from build123d import *

# Parameters (mm, degrees)
EXTRUDE1_DEPTH        = 78
M5_TAPPED_HOLE1_D     = 4.2
M5_TAPPED_HOLE1_DEPTH = 14.4
M5_TAPPED_HOLE1_TIP   = 1.2618073
SKETCH3_R             = 2.75
CUT_EXTRUDE1_DEPTH    = 93.649878575


with BuildPart() as part:
    # Sketch1 → Extrude1 (new, symmetric)
    with BuildSketch(Plane.XY):
        Polygon((0, 55), (0, 0), (30, 0), (30, 15), (15, 15), (15, 55), align=None)
    extrude(amount=EXTRUDE1_DEPTH, both=True)

    # M5 Tapped Hole1
    with Locations(Plane(origin=(7.5, 55, 0), x_dir=(0, 0, 1), z_dir=(0, 1, 0))):
        with Locations((0, 0), (-70, 0), (70, 0)):
            Hole(M5_TAPPED_HOLE1_D / 2, depth=M5_TAPPED_HOLE1_DEPTH)
            with Locations((0, 0, -(M5_TAPPED_HOLE1_DEPTH + M5_TAPPED_HOLE1_TIP / 2))):  # 118° drill point
                Cone(0, M5_TAPPED_HOLE1_D / 2, M5_TAPPED_HOLE1_TIP, mode=Mode.SUBTRACT)

    # Sketch3 → Cut-Extrude1 (cut, through all)
    with BuildSketch(Plane(origin=(0, 15, 0), x_dir=(1, 0, 0), z_dir=(0, 1, 0))):
        with Locations(Location((24, 0, 0), (0, 0, 270))):
            Circle(SKETCH3_R)
        with Locations(Location((24, 70, 0), (0, 0, 270))):
            Circle(SKETCH3_R)
        with Locations(Location((24, -70, 0), (0, 0, 90))):
            Circle(SKETCH3_R)
    extrude(amount=-CUT_EXTRUDE1_DEPTH, mode=Mode.SUBTRACT)


solid = part.part
CAD build for the part. Positions are in the model's coordinates, mm. A direction names the side the tool comes from. Give positions to 0.01 mm unless a question says otherwise; leave off trailing zeros. Write each loop counter-clockwise with the first axis right and the second up, starting at its lowest first coordinate (ties: lowest second). Pieces come first, ordered by that corner, then holes. Notation, with made-up numbers: (89.5, 35) - (115.5, 35) arc R35 ccw to (115.5, 71) - close; hole circle Ø2 at (-24, 62). An arc over 180 degrees is marked (long way). Answer as CSV lines item,"result".
Q1. Band-saw the part on A-A (y = 10). Give the cut face in (x, z), and give its area (3 significant figures).
Result set:
outline,"(0, -78) - (30, -78) - (30, 78) - (0, 78) - close; hole circle Ø5.5 at (24, -70); hole circle Ø5.5 at (24, 0); hole circle Ø5.5 at (24, 70)"
area,"4,610 mm²"
Q2. Drill centre lines: line 1 (Z direction, x = 7.5, y = 50.5); line 2 (X direction, y = 50.75, z = -70); line 3 (X direction, y = 52, z = 31). Where is each one in solid material? Low to high. Write a range as from..to.
Result set:
line 1,"-78..-72.1, -67.9..-2.1, 2.1..67.9, 72.1..78"
line 2,"0..5.4, 9.6..15"
line 3,"0..15"
Q3. Band-saw the part on C-C (y = 42). Give the cut face in (x, z).
Result set:
outline,"(0, -78) - (15, -78) - (15, 78) - (0, 78) - close; hole circle Ø4.2 at (7.5, -70); hole circle Ø4.2 at (7.5, 0); hole circle Ø4.2 at (7.5, 70)"
Q4. 3-axis set-ups, long thin cutter, end or side, ignore diameter. For faces 1 (the face through (9.582, 47.699, -69.727)), 2 (the face through (15, 35, 1)), 3 (the face through (11, 22, -78)): which of +Z, -Z, +X, -X, +Y, -Y reach the whole face in a straight line?
Result set:
face 1,"+Y"
face 2,"+Z, -Z, +X, +Y"
face 3,"-Z, +X, -X, +Y, -Y"
Q5. Band-saw the part on D-D (y = 21.5). Give the cut face in (x, z), and give its area (3 significant figures).
Result set:
outline,"(0, -78) - (15, -78) - (15, 78) - (0, 78) - close"
area,"2,340 mm²"
Q6. Band-saw the part on B-B (z = -10.5). Give the cut face in (x, y), and give its area (3 significant figures).
Result set:
outline,"(0, 0) - (30, 0) - (30, 15) - (15, 15) - (15, 55) - (0, 55) - close"
area,"1,050 mm²"
Q7. Pull direction X, two halves, no side cores. Call faces 4 (the face through (11, 55, 1)), 5 (the face through (7.81, 39.56, 0.2)), 6 (the face through (30, 7, 1)): released by +X, released by -X, zero draft, split by the parting line, or undercut.
Result set:
face 4,"zero draft"
face 5,"undercut"
face 6,"released by +X"
Q8. Flat gauge pins, fed straight in: pin 1 Ø5.5 at (x, z) = (7.5, 0) entering from -Y; pin 2 Ø2 at (y, z) = (41.5, 16) entering from +X; pin 3 Ø12 at (x, z) = (25.5, -36) entering from +Y; pin 4 Ø5 at (x, z) = (24, 0) entering from +Y. Where does each tip first touch, or does it go through?
Result set:
pin 1,"y = 0"
pin 2,"x = 15"
pin 3,"y = 15"
pin 4,"through"
